Check sheet for the modelled part. Datum: model origin and axes. Units: mm. A direction names the side the tool comes from. Round coordinates to 2 decimals unless told otherwise and drop trailing zeros. Order: outer loops, then holes, each group sorted by start corner. A loop starts at its lowest first (then second) coordinate and runs counter-clockwise, first axis right, second up. Notation, with made-up numbers: (2, 45.25) -> (42, 45.25) arc R26 ccw to (42, 62.25) -> close; hole circle Ø5 at (-5.5, 64). An arc over 180 degrees is marked (long way). Answer in a Markdown table with one row per item.
```python
from build123d import *

# Parameters (mm, degrees)
SKETCH2_R           = 17.5
SKETCH2_R_2         = 14.5
BOSS_EXTRUDE1_DEPTH = 15
BOSS_EXTRUDE2_DEPTH = 15
CHAMFER1_SIZE       = 0.5


with BuildPart() as part:
    # Sketch2 → Boss-Extrude1 (new body)
    with BuildSketch(Plane.XY):
        Circle(SKETCH2_R)
        Circle(SKETCH2_R_2, mode=Mode.SUBTRACT)
    extrude(amount=BOSS_EXTRUDE1_DEPTH)

    # Sketch4 → Boss-Extrude2 (add)
    with BuildSketch(Plane.XY):
        with BuildLine():
            Line((-1.5, 14.422205102), (-1, 12.961481397))
            ThreePointArc((-1, 12.961481397), (0, 13), (1, 12.961481397))
            Line((1, 12.961481397), (1.5, 14.422205102))
            ThreePointArc((1.5, 14.422205102), (0, 14.5), (-1.5, 14.422205102))
        make_face()
        with BuildLine():
            Line((1, -12.961481397), (1.5, -14.422205102))
            ThreePointArc((1.5, -14.422205102), (0, -14.5), (-1.5, -14.422205102))
            Line((-1.5, -14.422205102), (-1, -12.961481397))
            ThreePointArc((-1, -12.961481397), (0, -13), (1, -12.961481397))
        make_face()
    extrude(amount=BOSS_EXTRUDE2_DEPTH)

    # Chamfer1
    chamfer1_edges = [part.edges().sort_by_distance(p)[0] for p in [
        (-14.5, 0, 15),
        (-14.5, 0, 0),
        (-1.25, 13.691843249, 0),
        (0, 13, 0),
        (1.25, 13.691843249, 0),
        (1.25, 13.691843249, 15),
        (-1.25, 13.691843249, 15),
        (0, 13, 15),
        (14.5, 0, 0),
        (14.5, 0, 15),
        (1.25, -13.691843249, 0),
        (0, -13, 0),
        (-1.25, -13.691843249, 0),
        (-1.25, -13.691843249, 15),
        (1.25, -13.691843249, 15),
        (0, -13, 15),
    ]]
    chamfer(chamfer1_edges, length=CHAMFER1_SIZE)


solid = part.part
```
(1) Section check B-B on y = 0. Record the boundary of the cut face in (x, z), plus the area to 3 significant figures.
Solutions:
| item | result |
|---|---|
| outline | (-17.5, 0) -> (-15, 0) -> (-14.5, 0.5) -> (-14.5, 14.5) -> (-15, 15) -> (-17.5, 15) -> close; (14.5, 0.5) -> (15, 0) -> (17.5, 0) -> (17.5, 15) -> (15, 15) -> (14.5, 14.5) -> close |
| area | 89.5 mm^2 |
(2) Scan lines: probe 1 along X at (y, z) = (0.5, 9.25); probe 2 along Y at (x, z) = (0.5, 13); probe 3 along Y at (x, z) = (-7.5, 12.5). Record each from-to range of solid material in increasing order. Write a range as from..to.
Solutions:
| item | result |
|---|---|
| probe 1 | -17.49..-14.49, 14.49..17.49 |
| probe 2 | -17.49..-12.99, 12.99..17.49 |
| probe 3 | -15.81..-12.41, 12.41..15.81 |
(3) Section check A-A on x = 0. Record the boundary of the cut face in (y, z), plus the area to 4 significant figures.
Solutions:
| item | result |
|---|---|
| outline | (-17.5, 0) -> (-13.5, 0) -> (-13, 0.5) -> (-13, 14.5) -> (-13.5, 15) -> (-17.5, 15) -> close; (13, 0.5) -> (13.5, 0) -> (17.5, 0) -> (17.5, 15) -> (13.5, 15) -> (13, 14.5) -> close |
| area | 134.5 mm^2 |
(4) Tool access check on faces 1 (the flat face through (0, 14, 15)), 2 (the conical face through (14.632, 0.306, 14.635)), 3 (the flat face through (-1.08, 13.97, 0.25)), 4 (the cylindrical face through (14.497, -0.298, 7.402)). Record the directions out of +Z, -Z, +X, -X, +Y, -Y that give a thin tool (end or side, any length) a straight path to the whole face; none if there is none.
Solutions:
| item | result |
|---|---|
| face 1 | +Z, +X, -X, +Y, -Y |
| face 2 | +Z |
| face 3 | -Z |
| face 4 | +Z, -Z |
(5) Section check C-C on z = 2.5. Record the boundary of the cut face in (x, y), plus the area to 3 significant figures.
Solutions:
| item | result |
|---|---|
| outline | circle Ø35 at (0, 0); hole (-1.5, -14.42) -> (-1, -12.96) arc R13 ccw to (1, -12.96) -> (1.5, -14.42) arc R14.5 ccw to (1.5, 14.42) -> (1, 12.96) arc R13 ccw to (-1, 12.96) -> (-1.5, 14.42) arc R14.5 ccw to start |
| area | 309 mm^2 |
(6) Depth check by flat-ended pin: pin 1 Ø4 at (y, z) = (-6.5, 9) entering from +X; pin 2 Ø2 at (x, z) = (-12.5, 9.5) entering from +Y; pin 3 Ø8 at (x, z) = (8.5, 9.5) entering from -Y. Enter the tip coordinate at first touch or a pass-through.
Solutions:
| item | result |
|---|---|
| pin 1 | x = 16.91 |
| pin 2 | y = 13.19 |
| pin 3 | y = -16.91 |
(7) Draft check along Y on faces 5 (the cylindrical face through (-13.887, -10.648, 7.395)), 6 (the flat face through (0, 14, 0)), 7 (the flat face through (1.247, -13.682, 7.402)), 8 (the flat face through (1.076, -13.945, 14.747)). Enter one of: pulls with the +Y half, pulls with the -Y half, needs draft (parallel to the pull), parting line crosses it, or undercut.
Solutions:
| item | result |
|---|---|
| face 5 | parting line crosses it |
| face 6 | needs draft |
| face 7 | undercut |
| face 8 | undercut |
